```python
from build123d import *


with BuildPart() as part:
    # Bushing Profile Sketch → Bushing Body Revolve (revolve)
    with BuildSketch(Plane(origin=(0, 0, 0), x_dir=(0, 0, -1), z_dir=(1, 0, 0)), mode=Mode.PRIVATE) as bushing_body_revolve_sk:
        Polygon((0, 3.8), (-14, 3.8), (-14, 6), (-16, 6), (-16, 10), (-13, 10), (0, 7), align=None)
    revolve(bushing_body_revolve_sk.sketch.rotate(Axis((0, 0, 0), (0, 0, 1)), 90), axis=Axis((0, 0, 0), (0, 0, 1)))


solid = part.part
```
Verification items for the finished model (mm, model axes). A direction names the side the tool comes from. Coordinates: 2 decimals unless noted, no trailing zeros. Write each loop counter-clockwise with the first axis right and the second up, starting at its lowest first coordinate (ties: lowest second). Pieces come first, ordered by that corner, then holes. Notation, with made-up numbers: M 89.25,36.25 L 125.25,36.25 A19 ccw 125.25,59.25 Z; hole C -19,6.5 d8. An arc over 180 degrees is marked long. Answer as a JSON object with one key per item and string values. Group by question number.
(1) Cross-section at C-C, the plane z = 14.5. Record the cut outline in (x, y), and give its area (3 significant figures).
(2) Cross-section at A-A, the plane y = 0. Record the cut outline in (x, z), and give its area (3 significant figures).
(3) Release check for a two-part mould opening along Y. For faces 3 (the face through (0, 4, 14)), 4 (the face through (-3, 3, 0)), 5 (the face through (-7.77, -2.447, 4.965)) record: +Y half, -Y half, draft (parallel to the pull), parting line (faces both ways), or undercut.
(4) Gauge pin test, flat ends, axial feed: pin 1 (1.5 mm diameter, centred on y = 5, z = 5, fed in from +X); pin 2 (5 mm diameter, centred on x = 4, z = 4.5, fed in from +Y); pin 3 (3 mm diameter, centred on x = -2.5, z = 10, fed in from -Y). Record the tip position at first contact, or that the pin passes through.
(5) Tool access check on faces 1 (the face through (-5.723, -1.802, 15.014)), 2 (the face through (0, 7, 16)). Record the directions out of +Z, -Z, +X, -X, +Y, -Y that give a thin tool (end or side, any length) a straight path to the whole face; none if there is none.
(6) Cross-section at D-D, the plane z = 11.25. Record the cut outline in (x, y).
(7) Material ranges on line 1 (Y direction, x = 0, z = 14.8); line 2 (Y direction, x = -3.25, z = 3.5); line 3 (X direction, y = -2.5, z = 5), recorded low to high.
Reply:
{
 "1": {"outline": "C 0,0 d20; hole C 0,0 d12", "area": "201 mm²"},
 "2": {"outline": "M -10,13 L -7,0 L -3.8,0 L -3.8,14 L -6,14 L -6,16 L -10,16 Z; M 3.8,0 L 7,0 L 10,13 L 10,16 L 6,16 L 6,14 L 3.8,14 Z", "area": "151 mm²"},
 "3": {"face 3": "undercut", "face 4": "draft", "face 5": "parting line"},
 "4": {"pin 1": "x = 7", "pin 2": "y = 8.15", "pin 3": "y = -9.45"},
 "5": {"face 1": "+Z", "face 2": "+Z, +X, -X, +Y, -Y"},
 "6": {"outline": "C 0,0 d19.19; hole C 0,0 d7.6"},
 "7": {"line 1": "-10 to -6, 6 to 10", "line 2": "-7.1 to -1.97, 1.97 to 7.1", "line 3": "-7.76 to -2.86, 2.86 to 7.76"}
}
